Design review of the part shown in the three views and the two pictorial views. Dimensions are in mm from the part's minimum x, y and z. Give positions to 0.01 mm unless a question says otherwise; leave off trailing zeros. Loops run counter-clockwise (first coordinate to the right, second up) from the corner with the lowest first, then second, coordinate; pieces in that order, holes last. Notation, with made-up numbers: (37.5, 32) - (41.5, 32) arc R23 cw to (41.5, 56) - close; hole circle Ø11 at (79.5, -30.5). An arc over 180 degrees is marked (long way). Answer in a Markdown table with one row per item.
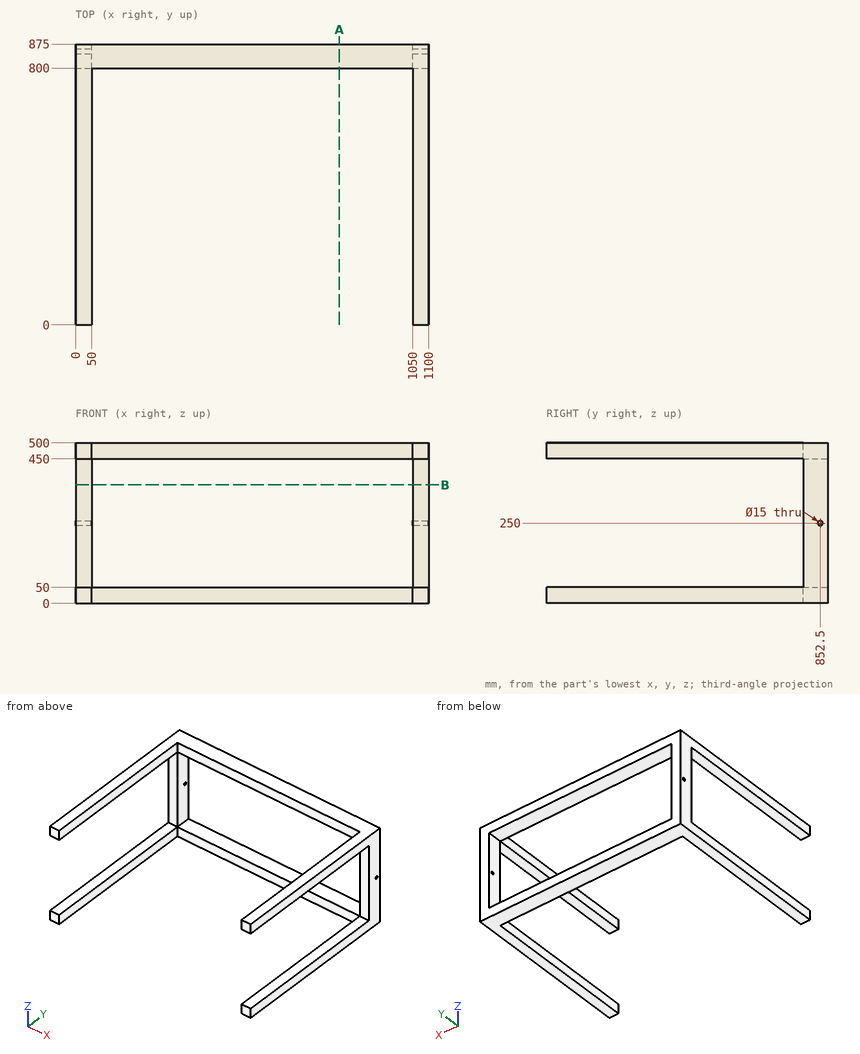
1. Wall thickness on line 1 (X direction, y = 103, z = 471.5); line 2 (Y direction, x = 1080.5, z = 250); line 3 (Z direction, x = 15, y = 852.5): over which ranges is each line inside the solid? List them lowest first. Write a range as [from, to].
Values:
| item | result |
|---|---|
| line 1 | x = [0, 50], [1050, 1100] |
| line 2 | y = [800, 845], [860, 875] |
| line 3 | z = [0, 242.5], [257.5, 500] |
2. Clearance check with flat-ended pins moving along their axes: pin 1 (25 mm diameter, centred on y = 386, z = 477.5, fed in from -X); pin 2 (9 mm diameter, centred on y = 852.5, z = 250, fed in from -X) (3 decimals); pin 3 (25 mm diameter, centred on x = 380, z = 479.5, fed in from -Y). State where each tip first meets the part, or that it passes through.
Values:
| item | result |
|---|---|
| pin 1 | stops at x = 0 |
| pin 2 | passes through |
| pin 3 | stops at y = 800 |
3. We need section B-B, the plane z = 369. Give the boundary of the cut face in (x, y).
Values:
| item | result |
|---|---|
| outline | (0, 800) - (50, 800) - (50, 875) - (0, 875) - close; (1050, 800) - (1100, 800) - (1100, 875) - (1050, 875) - close |
4. We need section A-A, the plane x = 822. Give the boundary of the cut face in (y, z).
Values:
| item | result |
|---|---|
| outline | (800, 0) - (875, 0) - (875, 50) - (800, 50) - close; (800, 450) - (875, 450) - (875, 500) - (800, 500) - close |
